For this review, use the dimensioned drawing (mm, ordinates from the lowest corner) and the shaded views. A direction names the side the tool comes from. Coordinates: 2 decimals unless noted, no trailing zeros. Write each loop counter-clockwise with the first axis right and the second up, starting at its lowest first coordinate (ties: lowest second). Pieces come first, ordered by that corner, then holes.
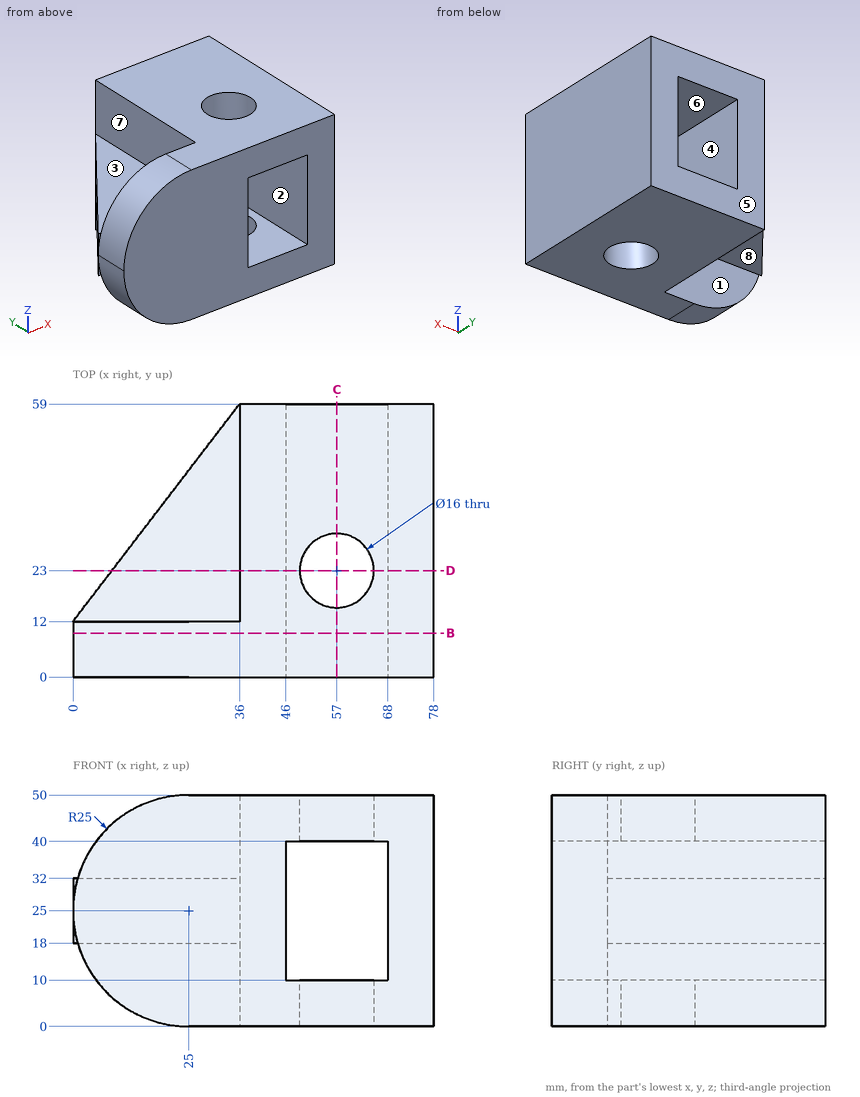
Item 1: For pin 1 (5 mm diameter, centred on x = 11, y = 9, fed in from +Z); pin 2 (5.5 mm diameter, centred on x = 23, z = 9.5, fed in from +Y); pin 3 (9.5 mm diameter, centred on x = 57, y = 23, fed in from +Z); pin 4 (4 mm diameter, centred on y = 6.5, z = 19, fed in from -X), all flat-tipped, find the tip position at first contact; note any pin that passes through.
Solved:
pin 1: stops at z = 47.2
pin 2: stops at y = 12
pin 3: passes through
pin 4: stops at x = 0.32
Item 2: Machinability: for the marked faces 5, 6, 7 and 8, which of the approach directions +Z, -Z, +X, -X, +Y, -Y give a long, thin tool a straight path to every point of the face, cutting with its end or side? Answer none if there is none.
Solved:
face 5: +Z, -Z, +X, -X, +Y
face 6: +Y, -Y
face 7: +Z, -X, +Y
face 8: -Z, -X, +Y
Item 3: Take a section at B-B, the plane y = 9.5. Write out the cut boundary in (x, z), plus the area to 3 significant figures.
Solved:
outline: (25, 0) - (78, 0) - (78, 50) - (25, 50) arc R25 ccw to start; hole (46, 10) - (68, 10) - (68, 40) - (46, 40) - close
area: 2,970 mm2
Item 4: Take a section at D-D, the plane y = 23. Write out the cut boundary in (x, z).
Solved:
outline: (8.43, 18) - (36, 18) - (36, 0) - (49, 0) - (49, 10) - (46, 10) - (46, 40) - (49, 40) - (49, 50) - (36, 50) - (36, 32) - (8.43, 32) - close; (65, 0) - (78, 0) - (78, 50) - (65, 50) - (65, 40) - (68, 40) - (68, 10) - (65, 10) - close
Item 5: Mouldability with a two-part tool opening along Z and no side actions: class the marked faces 1, 2, 3 and 4 as pulls with the +Z half, pulls with the -Z half, needs draft (parallel to the pull), parting line crosses it, or undercut.
Solved:
face 1: needs draft
face 2: undercut
face 3: pulls with the +Z half
face 4: undercut
Item 6: To check wall thickness, follow line 1 along Z through (x, y) = (61.5, 42.5); line 2 along Y through (x, z) = (57, 3.5); line 3 along X through (y, z) = (41, 25). State the ranges of each line that lie inside material, in increasing order.
Solved:
line 1: z = 0 to 10, 40 to 50
line 2: y = 0 to 15, 31 to 59
line 3: x = 22.21 to 46, 68 to 78
Item 7: Take a section at C-C, the plane x = 57. Write out the cut boundary in (y, z).
Solved:
outline: (0, 0) - (15, 0) - (15, 10) - (0, 10) - close; (0, 40) - (15, 40) - (15, 50) - (0, 50) - close; (31, 0) - (59, 0) - (59, 10) - (31, 10) - close; (31, 40) - (59, 40) - (59, 50) - (31, 50) - close
